Part model, mm, in its own coordinate system. Coordinates: 2 decimals unless noted, no trailing zeros. Loops run counter-clockwise (first coordinate to the right, second up) from the corner with the lowest first, then second, coordinate; pieces in that order, holes last. Notation, with made-up numbers: (14.25, 69.5) - (46.25, 69.5) arc R26 ccw to (46.25, 108.5) - close; hole circle Ø10 at (66, 15.25). An arc over 180 degrees is marked (long way). Use a Markdown table: item, result. Add a question column.
1) Band-saw the part on A-A (z = -1037.25). Give the cut face in (x, y).
2) Drop flat-ended pins along their axis: P1, Ø5, axis at x = -12.5, z = -1038, coming from the +Y side; P2, Ø6, axis at x = -3, z = -1036, coming from the -Y side; P3, Ø1, axis at y = 472.5, z = -1040, coming from the -X side. Give the stop position or say it passes through.
3) Probe probe 1 along Y at (x, z) = (-145.5, -1042.5); probe 2 along Y at (x, z) = (-128.5, -1037); probe 3 along Y at (x, z) = (-124, -1040). List the from-to ranges inside material, lowest first. Write a range as [from, to].
4) Band-saw the part on C-C (x = 117.5). Give the cut face in (y, z), plus the area to 3 significant figures.
5) Band-saw the part on B-B (y = 442.5). Give the cut face in (x, z).
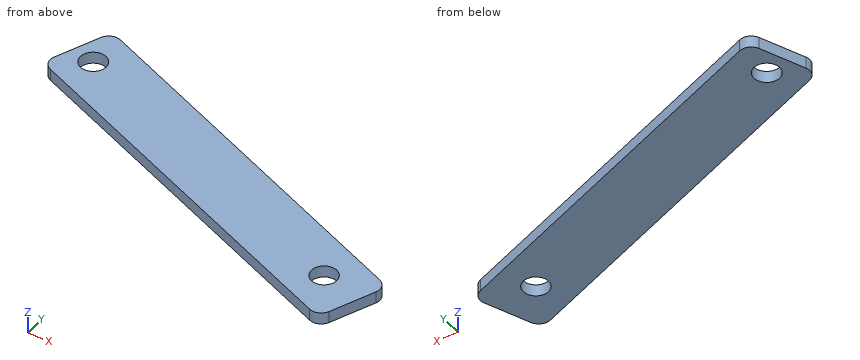
from build123d import *

# Parameters (mm, degrees)
EXTRUDE_START   = 40
SKETCH_1_R      = 11
SKETCH_1_R_2    = 10.824525282
EXTRUDE_1_DEPTH = 10


with BuildPart() as part:
    # 草图1 → 凸台-拉伸1 (new body)
    with BuildSketch(Plane.XY.offset(-1083.237354735).offset(EXTRUDE_START)):
        with BuildLine():
            Line((-135.515744069, 493.626345969), (171.40128741, 372.374806646))
            ThreePointArc((171.40128741, 372.374806646), (176.901571064, 367.052633829), (177.027514445, 359.40000147))
            Line((177.027514445, 359.40000147), (162.330358163, 322.197937048))
            ThreePointArc((162.330358163, 322.197937048), (157.008185347, 316.697653394), (149.355552988, 316.571710013))
            Line((149.355552988, 316.571710013), (-157.561478491, 437.823249336))
            ThreePointArc((-157.561478491, 437.823249336), (-163.061762145, 443.145422153), (-163.187705526, 450.798054512))
            Line((-163.187705526, 450.798054512), (-148.490549245, 488.000118934))
            ThreePointArc((-148.490549245, 488.000118934), (-143.168376428, 493.500402588), (-135.515744069, 493.626345969))
        make_face()
        with Locations((-137.238095175, 462.050508582)):
            Circle(SKETCH_1_R, mode=Mode.SUBTRACT)
        with Locations((136.038969551, 354.088872827)):
            Circle(SKETCH_1_R_2, mode=Mode.SUBTRACT)
    extrude(amount=EXTRUDE_1_DEPTH)


solid = part.part
Answer block:
| question | item | result |
|---|---|---|
| 1 | outline | (-163.19, 450.8) arc R10 ccw to (-157.56, 437.82) - (149.36, 316.57) arc R10 ccw to (162.33, 322.2) - (177.03, 359.4) arc R10 ccw to (171.4, 372.37) - (-135.52, 493.63) arc R10 ccw to (-148.49, 488) - close; hole circle Ø22 at (-137.24, 462.05); hole circle Ø21.65 at (136.04, 354.09) |
| 2 | P1 | y = 446.02 |
| 2 | P2 | y = 375.58 |
| 2 | P3 | x = -154.81 |
| 3 | probe 1 | [433.06, 454.79], [469.31, 492.08] |
| 3 | probe 2 | [426.34, 455.37], [468.73, 490.85] |
| 3 | probe 3 | [424.56, 489.08] |
| 4 | outline | (329.16, -1043.24) - (393.67, -1043.24) - (393.67, -1033.24) - (329.16, -1033.24) - close |
| 4 | area | 645 mm2 |
| 5 | outline | (-162.75, -1043.24) - (-6.1, -1043.24) - (-6.1, -1033.24) - (-162.75, -1033.24) - close |
